For this review, take the finished solid that the model builds, in its own axes (mm). Round coordinates to 2 decimals unless told otherwise and drop trailing zeros. Loops run counter-clockwise (first coordinate to the right, second up) from the corner with the lowest first, then second, coordinate; pieces in that order, holes last. Notation, with made-up numbers: (-3, 28) -> (16, 28) arc R8 ccw to (16, 37) -> close; hole circle Ø10 at (11, -6). An arc over 180 degrees is marked (long way). Write each question's results on one line, items separated by ' | '.
```python
from build123d import *

# Parameters (mm, degrees)
SKETCH_1_W          = 296
SKETCH_1_H          = 267.5
EXTRUDE_1_DEPTH     = 1.5
FILLET_1_R          = 3
SKETCH_6_R          = 3
CUT_EXTRUDE_1_DEPTH = 1.5
SKETCH_7_R          = 3.55
CUT_EXTRUDE_2_DEPTH = 1.5
CHAMFER_1_SIZE      = 1


with BuildPart() as part:
    # 草图1 → 凸台-拉伸1 (new body)
    with BuildSketch(Plane.XY):
        with Locations((-237.5, 200.75)):
            Rectangle(SKETCH_1_W, SKETCH_1_H)
    extrude(amount=-EXTRUDE_1_DEPTH)

    # 圆角1
    fillet_1_edges = [part.edges().sort_by_distance(p)[0] for p in [
        (-385.5, 67, -0.75),
        (-385.5, 334.5, -0.75),
        (-89.5, 334.5, -0.75),
        (-89.5, 67, -0.75),
    ]]
    fillet(fillet_1_edges, radius=FILLET_1_R)

    # 草图6 → 切除-拉伸1 (cut)
    with BuildSketch(Plane.XY):
        with Locations((-367, 91.5)):
            Circle(SKETCH_6_R)
        with Locations((-187, 91.5)):
            Circle(SKETCH_6_R)
    extrude(amount=-CUT_EXTRUDE_1_DEPTH, mode=Mode.SUBTRACT)

    # 草图7 → 切除-拉伸2 (cut)
    with BuildSketch(Plane(origin=(0, 0, -1.5), x_dir=(-1, 0, 0), z_dir=(0, 0, -1))):
        with Locations((98, 326)):
            Circle(SKETCH_7_R)
        with Locations((377, 326)):
            Circle(SKETCH_7_R)
        with Locations((377, 75.5)):
            Circle(SKETCH_7_R)
        with Locations((98, 75.5)):
            Circle(SKETCH_7_R)
    extrude(amount=-CUT_EXTRUDE_2_DEPTH, mode=Mode.SUBTRACT)

    # 倒角1
    chamfer_1_edges = [part.edges().sort_by_distance(p)[0] for p in [
        (-94.45, 326, -1.5),
        (-373.45, 326, -1.5),
        (-373.45, 75.5, -1.5),
        (-94.45, 75.5, -1.5),
    ]]
    chamfer(chamfer_1_edges, length=CHAMFER_1_SIZE)


solid = part.part
```
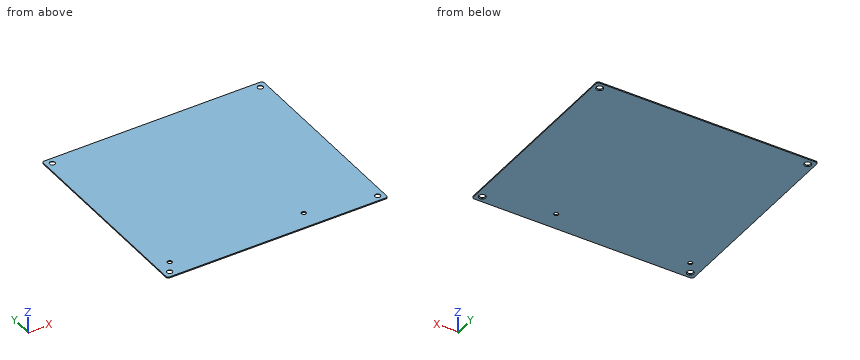
1. Consider section B-B (x = -98). State the section outline as (y, z) points.
Values found:
outline: (67, -1.5) -> (70.95, -1.5) -> (71.95, -0.5) -> (71.95, 0) -> (67, 0) -> close; (79.05, -0.5) -> (80.05, -1.5) -> (321.45, -1.5) -> (322.45, -0.5) -> (322.45, 0) -> (79.05, 0) -> close; (329.55, -0.5) -> (330.55, -1.5) -> (334.5, -1.5) -> (334.5, 0) -> (329.55, 0) -> close
2. To check wall thickness, follow probe 1 along Y at (x, z) = (-98, -0.15); probe 2 along X at (y, z) = (326, -0.3); probe 3 along Y at (x, z) = (-187, -0.25). State the ranges of each line that lie inside material, in increasing order.
Values found:
probe 1: y = 67 to 71.95, 79.05 to 322.45, 329.55 to 334.5 | probe 2: x = -385.5 to -380.55, -373.45 to -101.55, -94.45 to -89.5 | probe 3: y = 67 to 88.5, 94.5 to 334.5
3. For pin 1 (8 mm diameter, centred on x = -98, y = 75.5, fed in from -Z), flat-tipped, find the tip position at first contact; note if it passes through.
Values found:
pin 1: stops at z = -0.95
4. Consider section A-A (y = 75.5). State the section outline as (x, z) points.
Values found:
outline: (-385.5, -1.5) -> (-381.55, -1.5) -> (-380.55, -0.5) -> (-380.55, 0) -> (-385.5, 0) -> close; (-373.45, -0.5) -> (-372.45, -1.5) -> (-102.55, -1.5) -> (-101.55, -0.5) -> (-101.55, 0) -> (-373.45, 0) -> close; (-94.45, -0.5) -> (-93.45, -1.5) -> (-89.5, -1.5) -> (-89.5, 0) -> (-94.45, 0) -> close
